from build123d import *

# Parameters (mm, degrees)
SKETCH1_W                                            = 85
SKETCH1_H                                            = 10
BOSS_EXTRUDE1_DEPTH                                  = 10
CUT_EXTRUDE1_DEPTH                                   = 4.4
CUT_EXTRUDE2_DEPTH                                   = 45.018291652
SKETCH4_W                                            = 9.4
SKETCH4_H                                            = 10
BOSS_EXTRUDE2_DEPTH                                  = 10
SKETCH5_W                                            = 10
SKETCH5_H                                            = 10
CUT_EXTRUDE3_DEPTH                                   = 5
M6_TAPPED_HOLE1_D                                    = 5
M6_TAPPED_HOLE1_DEPTH                                = 5
M6_TAPPED_HOLE1_TIP                                  = 1.502151548
CBORE_FOR_M4_HEXAGON_SOCKET_HEAD_CAP_SCR_D           = 4.5
CBORE_FOR_M4_HEXAGON_SOCKET_HEAD_CAP_SCR_DEPTH       = 14
CBORE_FOR_M4_HEXAGON_SOCKET_HEAD_CAP_SCR_CBORE_D     = 8
CBORE_FOR_M4_HEXAGON_SOCKET_HEAD_CAP_SCR_CBORE_DEPTH = 4.6
CBORE_FOR_M4_HEXAGON_SOCKET_HEAD_CAP_SCR_TIP         = 1.351936393
FILLET1_R                                            = 3
FILLET2_R                                            = 1
CHAMFER1_SIZE                                        = 1


with BuildPart() as part:
    # Sketch1 → Boss-Extrude1 (new body)
    with BuildSketch(Plane(origin=(0, 0, 0), x_dir=(1, 0, 0), z_dir=(0, 1, 0))):
        Rectangle(SKETCH1_W, SKETCH1_H)
    extrude(amount=BOSS_EXTRUDE1_DEPTH)

    # Sketch2 → Cut-Extrude1 (cut)
    with BuildSketch(Plane.XY.offset(-5)):
        with BuildLine():
            Line((-27.75, 9), (27.75, 9))
            ThreePointArc((27.75, 9), (31.75, 5), (27.75, 1))
            Line((27.75, 1), (-27.75, 1))
            ThreePointArc((-27.75, 1), (-31.75, 5), (-27.75, 9))
        make_face()
    extrude(amount=CUT_EXTRUDE1_DEPTH, mode=Mode.SUBTRACT)

    # Sketch3 → Cut-Extrude2 (cut, through all)
    with BuildSketch(Plane(origin=(0, 0, -0.6), x_dir=(-1, 0, 0), z_dir=(0, 0, -1))):
        with BuildLine():
            Line((-27.75, 7.25), (27.75, 7.25))
            ThreePointArc((27.75, 7.25), (30, 5), (27.75, 2.75))
            Line((27.75, 2.75), (-27.75, 2.75))
            ThreePointArc((-27.75, 2.75), (-30, 5), (-27.75, 7.25))
        make_face()
    extrude(amount=-CUT_EXTRUDE2_DEPTH, mode=Mode.SUBTRACT)

    # Sketch4 → Boss-Extrude2 (add)
    with BuildSketch(Plane.XY.offset(-5)):
        with Locations((-37.8, 5)):
            Rectangle(SKETCH4_W, SKETCH4_H)
    extrude(amount=-BOSS_EXTRUDE2_DEPTH)

    # Sketch5 → Cut-Extrude3 (cut)
    with BuildSketch(Plane.XY.offset(5)):
        with Locations((37.5, 5)):
            Rectangle(SKETCH5_W, SKETCH5_H)
    extrude(amount=-CUT_EXTRUDE3_DEPTH, mode=Mode.SUBTRACT)

    # M6 Tapped Hole1
    with Locations(Plane(origin=(0, 0, -15), x_dir=(-1, 0, 0), z_dir=(0, 0, -1))):
        with Locations((37.8, 4.802472567)):
            Hole(M6_TAPPED_HOLE1_D / 2, depth=M6_TAPPED_HOLE1_DEPTH)
            with Locations((0, 0, -(M6_TAPPED_HOLE1_DEPTH + M6_TAPPED_HOLE1_TIP / 2))):  # 118° drill point
                Cone(0, M6_TAPPED_HOLE1_D / 2, M6_TAPPED_HOLE1_TIP, mode=Mode.SUBTRACT)

    # CBORE for M4 Hexagon socket head cap screws1
    with Locations(Plane(origin=(0, 0, -5), x_dir=(-1, 0, 0), z_dir=(0, 0, -1))):
        with Locations((-37.5, 5.5)):
            CounterBoreHole(CBORE_FOR_M4_HEXAGON_SOCKET_HEAD_CAP_SCR_D / 2, CBORE_FOR_M4_HEXAGON_SOCKET_HEAD_CAP_SCR_CBORE_D / 2, CBORE_FOR_M4_HEXAGON_SOCKET_HEAD_CAP_SCR_CBORE_DEPTH, depth=CBORE_FOR_M4_HEXAGON_SOCKET_HEAD_CAP_SCR_DEPTH)
            with Locations((0, 0, -(CBORE_FOR_M4_HEXAGON_SOCKET_HEAD_CAP_SCR_DEPTH + CBORE_FOR_M4_HEXAGON_SOCKET_HEAD_CAP_SCR_TIP / 2))):  # 118° drill point
                Cone(0, CBORE_FOR_M4_HEXAGON_SOCKET_HEAD_CAP_SCR_D / 2, CBORE_FOR_M4_HEXAGON_SOCKET_HEAD_CAP_SCR_TIP, mode=Mode.SUBTRACT)

    # Fillet1
    fillet1_edges = [part.edges().sort_by_distance(p)[0] for p in [
        (42.5, 0, -2.5),
        (42.5, 10, -2.5),
        (32.5, 0, 2.5),
        (32.5, 10, 2.5),
    ]]
    fillet(fillet1_edges, radius=FILLET1_R)

    # Fillet2
    fillet2_edges = [part.edges().sort_by_distance(p)[0] for p in [
        (-33.1, 5, -5),
    ]]
    fillet(fillet2_edges, radius=FILLET2_R)

    # Chamfer1
    chamfer1_edges = [part.edges().sort_by_distance(p)[0] for p in [
        (-37.8, 0, -15),
        (-42.5, 5, -15),
        (-37.8, 10, -15),
        (-33.1, 5, -15),
        (-42.5, 10, -5),
        (-6.5, 0, 5),
        (-42.5, 0, -5),
        (-42.5, 5, 5),
        (-6.5, 10, 5),
        (32.5, 5, 5),
        (31.621320344, 9.121320344, 5),
        (31.621320344, 0.878679656, 5),
    ]]
    chamfer(chamfer1_edges, length=CHAMFER1_SIZE)


solid = part.part
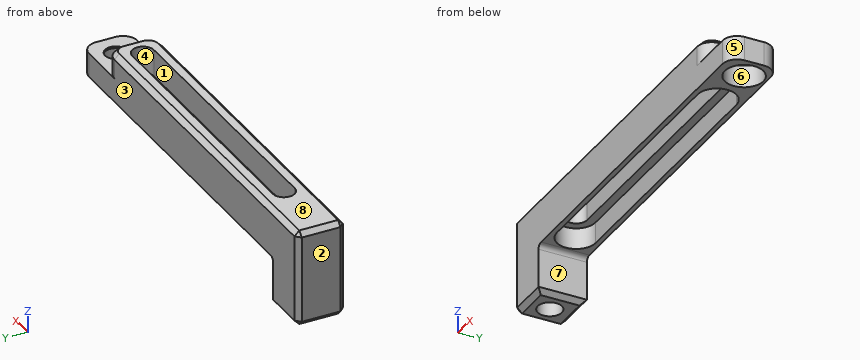
Here's how the part is built. I have some questions about the finished solid (model axes, mm). Face numbers are marked on the shaded views. A direction names the side the tool comes from. Round coordinates to 2 decimals unless told otherwise and drop trailing zeros. Order: outer loops, then holes, each group sorted by start corner. A loop starts at its lowest first (then second) coordinate and runs counter-clockwise, first axis right, second up. Notation, with made-up numbers: (62.25, -29) -> (102.25, -29) arc R16 ccw to (102.25, -5) -> close; hole circle Ø9 at (14, -23.75). An arc over 180 degrees is marked (long way). Return JSON: item names as keys, results as strings.
Q1. Which directions (+Z, -Z, +X, -X, +Y, -Y) give clear straight access to the entire face, cutting with the end or side of a thin tool? Please do the marked faces 4, 5, 6, 7 and 8.
Filled sheet:
{"face 4": "+Z, -Z", "face 5": "+Z, -Z, +X, -Y", "face 6": "-Z", "face 7": "-Z, +X, +Y, -Y", "face 8": "+Z, +X, -X, +Y, -Y"}
Q2. If we mould it in two halves opening along Y, with no side actions, what happens to the marked faces 1, 2 and 3? For each: released by +Y, released by -Y, zero draft, split by the parting line, or undercut.
Filled sheet:
{"face 1": "undercut", "face 2": "zero draft", "face 3": "released by +Y"}
Q3. For pin 1 Ø5 at (x, y) = (37.5, 5.5) entering from +Z; pin 2 Ø1 at (x, y) = (-28, 4.5) entering from -Z; pin 3 Ø3 at (x, y) = (5.5, 6.5) entering from -Z; pin 4 Ø2.5 at (y, z) = (6.5, -8.5) entering from +X, each with a flat end and sliding along its axis, tell me the tip position at first contact or that it passes through.
Filled sheet:
{"pin 1": "stops at z = 0", "pin 2": "passes through", "pin 3": "stops at z = -0.6", "pin 4": "stops at x = -33.1"}
Q4. If we section it at A-A on x = 8: List the corners of the cut face in (y, z) for me.
Filled sheet:
{"outline": "(0, -5) -> (1, -5) -> (1, -0.6) -> (2.75, -0.6) -> (2.75, 5) -> (1, 5) -> (0, 4) -> close; (7.25, -0.6) -> (9, -0.6) -> (9, -5) -> (10, -5) -> (10, 4) -> (9, 5) -> (7.25, 5) -> close"}
Q5. I need wall thicknesses on line 1 along X through (y, z) = (5, -0.75); line 2 along Y through (x, z) = (3, -2.5); line 3 along Y through (x, z) = (37.5, -2.2). Which ranges of each line are inside material? Lowest first, please. Write a range as from..to.
Filled sheet:
{"line 1": "x = -42.5..-31.75, 31.75..33.53, 41.47..42.5", "line 2": "y = 0..1, 9..10", "line 3": "y = 0..1.5, 9.5..10"}
Q6. If we section it at B-B on z = -10.75: List the corners of the cut face in (x, y) for me, plus the area to 3 significant figures.
Filled sheet:
{"outline": "(-42.5, 1) -> (-41.5, 0) -> (-33.1, 0) -> (-33.1, 10) -> (-41.5, 10) -> (-42.5, 9) -> close; hole circle Ø5 at (-37.8, 4.8)", "area": "73.4 mm^2"}
